Model file for the job. Use its own axes, mm. A direction names the side the tool comes from. Give positions to 0.01 mm unless a question says otherwise; leave off trailing zeros. Write each loop counter-clockwise with the first axis right and the second up, starting at its lowest first coordinate (ties: lowest second). Pieces come first, ordered by that corner, then holes. Notation, with made-up numbers: M 7,47 L 64,47 A7 ccw 64,51 Z; hole C 14.5,47 d8. An arc over 180 degrees is marked long. Answer as a JSON object with one key per item and string values. Group by question number.
```python
from build123d import *

# Parameters (mm, degrees)
SKETCH1_W             = 75
SKETCH1_H             = 60
BOSS_EXTRUDE1_DEPTH   = 6
CUT_EXTRUDE1_DEPTH    = 50.5
M6_TAPPED_HOLE1_D     = 5
M6_TAPPED_HOLE1_DEPTH = 12
M6_TAPPED_HOLE1_TIP   = 1.502151548
M6_TAPPED_HOLE2_D     = 5
M6_TAPPED_HOLE2_DEPTH = 15
M6_TAPPED_HOLE2_TIP   = 1.502151548
CHAMFER1_SIZE         = 1


with BuildPart() as part:
    # Sketch1 → Boss-Extrude1 (new, symmetric)
    with BuildSketch(Plane.XY):
        Rectangle(SKETCH1_W, SKETCH1_H)
    extrude(amount=BOSS_EXTRUDE1_DEPTH, both=True)

    # Sketch2 → Cut-Extrude1 (cut, through all)
    with BuildSketch(Plane.XY.offset(6)):
        Polygon((-27.5, 30), (37.5, -20), (37.5, 30), align=None)
    extrude(amount=-CUT_EXTRUDE1_DEPTH, mode=Mode.SUBTRACT)

    # M6 Tapped Hole1
    with Locations(Plane.ZY.offset(37.5)):
        with Locations((0, 20), (0, -15)):
            Hole(M6_TAPPED_HOLE1_D / 2, depth=M6_TAPPED_HOLE1_DEPTH)
            with Locations((0, 0, -(M6_TAPPED_HOLE1_DEPTH + M6_TAPPED_HOLE1_TIP / 2))):  # 118° drill point
                Cone(0, M6_TAPPED_HOLE1_D / 2, M6_TAPPED_HOLE1_TIP, mode=Mode.SUBTRACT)

    # M6 Tapped Hole2
    with Locations(Plane(origin=(0, -30, 0), x_dir=(-1, 0, 0), z_dir=(0, -1, 0))):
        with Locations((22.5, 0), (-27.5, 0)):
            Hole(M6_TAPPED_HOLE2_D / 2, depth=M6_TAPPED_HOLE2_DEPTH)
            with Locations((0, 0, -(M6_TAPPED_HOLE2_DEPTH + M6_TAPPED_HOLE2_TIP / 2))):  # 118° drill point
                Cone(0, M6_TAPPED_HOLE2_D / 2, M6_TAPPED_HOLE2_TIP, mode=Mode.SUBTRACT)

    # Chamfer1
    chamfer1_edges = [part.edges().sort_by_distance(p)[0] for p in [
        (37.5, -30, 0),
        (-37.5, -30, 0),
        (-37.5, 30, 0),
    ]]
    chamfer(chamfer1_edges, length=CHAMFER1_SIZE)


solid = part.part
```
Q1. Slice it at A-A, the plane x = -32. Write the cut outline in (y, z).
Q2. Two-plate mould, pull along Z, no slides. Class faces 1 (the flat face through (5, 5, 0)), 2 (the flat face through (-9, -6, 6)), 3 (the conical face through (-22.066, -13.759, -0.019)): +Z half, -Z half, draft (parallel to the pull), parting line (faces both ways), or undercut.
Q3. Slice it at C-C, the plane x = 12.5. Write the cut outline in (y, z), then the cut area to 3 significant figures.
Q4. 3-axis set-ups, long thin cutter, end or side, ignore diameter. For faces 4 (the cylindrical face through (-20.19, -22.4, 0.96)), 5 (the cylindrical face through (-31.42, -17.44, 0.54)), 6 (the flat face through (-1, -30, 0)): which of +Z, -Z, +X, -X, +Y, -Y reach the whole face in a straight line?
Q5. Slice it at B-B, the plane y = 11. Write the cut outline in (x, z), then the cut area to 3 significant figures.
Q6. Wall check: L1, parallel to Y at x = -33.75, z = 0; L2, parallel to Z at x = -35, y = 20; L3, parallel to Z at x = 27, y = -22. Give the ranges that are in metal, low to high.
Q7. Drop flat-ended pins along their axis: P1, Ø1.5, axis at x = -23.5, z = 2.5, coming from the +Y side; P2, Ø4, axis at y = 20, z = 0, coming from the +X side; P3, Ø4, axis at x = -22.5, z = 0, coming from the +Y side. Give the stop position or say it passes through.
Solved:
{
 "1": {"outline": "M -30,-6 L 30,-6 L 30,6 L -30,6 Z; hole C -15,0 d5; hole C 20,0 d5"},
 "2": {"face 1": "draft", "face 2": "+Z half", "face 3": "undercut"},
 "3": {"outline": "M -30,-6 L -0.77,-6 L -0.77,6 L -30,6 Z", "area": "351 mm²"},
 "4": {"face 4": "-Y", "face 5": "-X", "face 6": "+Z, -Z, +X, -X, -Y"},
 "5": {"outline": "M -37.5,-6 L -2.8,-6 L -2.8,6 L -37.5,6 Z", "area": "416 mm²"},
 "6": {"L1": "y = -30 to -17.5, -12.5 to 17.5, 22.5 to 30", "L2": "z = -6 to -2.5, 2.5 to 6", "L3": "z = -6 to -2.45, 2.45 to 6"},
 "7": {"P1": "stops at y = 27.5", "P2": "stops at x = -11.9", "P3": "stops at y = 27.69"}
}
